Job drawing, mm, ordinate dimensions from the low corner. One solid piece. A direction names the side the tool comes from. Give positions to 0.01 mm unless a question says otherwise; leave off trailing zeros. Order: outer loops, then holes, each group sorted by start corner. A loop starts at its lowest first (then second) coordinate and runs counter-clockwise, first axis right, second up. Notation, with made-up numbers: (-13, 29) - (37, 29) arc R20 cw to (37, 49) - close; hole circle Ø8 at (-37, 6). An arc over 180 degrees is marked (long way). One line per item, written item: value.
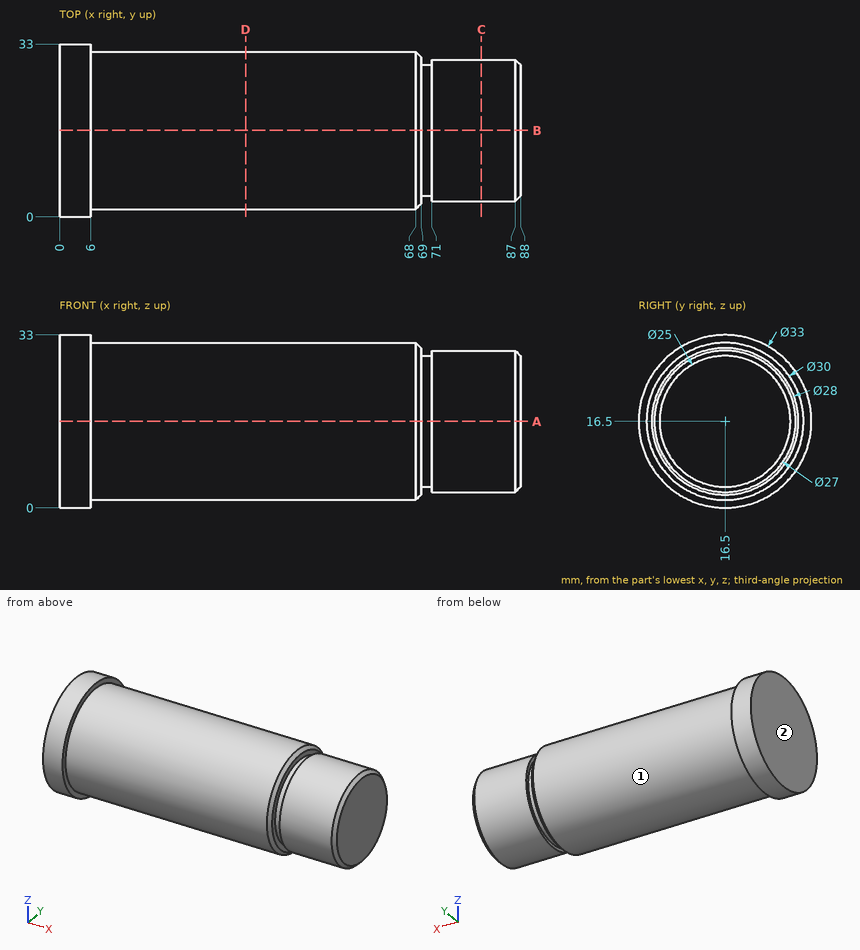
1) Slice it at C-C on x = 80.5. Write the cut outline in (y, z).
Answer:
outline: circle Ø27 at (16.5, 16.5)
2) Slice it at A-A on z = 16.5. Write the cut outline in (x, y).
Answer:
outline: (0, 0) - (6, 0) - (6, 1.5) - (68, 1.5) - (69, 2.5) - (69, 4) - (71, 4) - (71, 3) - (87, 3) - (88, 4) - (88, 29) - (87, 30) - (71, 30) - (71, 29) - (69, 29) - (69, 30.5) - (68, 31.5) - (6, 31.5) - (6, 33) - (0, 33) - close
3) Which spindle directions (+Z, -Z, +X, -X, +Y, -Y) get a long thin tool onto all of the face, cutting with end or side? Do the marked faces 1 and 2. Say none if no direction does.
Answer:
face 1: +X
face 2: +Z, -Z, -X, +Y, -Y
4) Wall check: line 1 along Y through (x, z) = (78.5, 16); line 2 along Y through (x, z) = (15.5, 17); line 3 along Z through (x, y) = (50, 17.5). Give the ranges that are in metal, low to high. Write a range as [from, to].
Answer:
line 1: y = [3.01, 29.99]
line 2: y = [1.51, 31.49]
line 3: z = [1.53, 31.47]
5) Slice it at D-D on x = 35.5. Write the cut outline in (y, z).
Answer:
outline: circle Ø30 at (16.5, 16.5)
6) Drop flat-ended pins along their axis: P1, Ø8, axis at x = 45.5, y = 20.5, coming from the +Z side; P2, Ø2, axis at x = 20, y = 18.5, coming from the -Z side; P3, Ø2, axis at x = 16, z = 24.5, coming from the +Y side. Give the stop position or say it passes through.
Answer:
P1: stops at z = 31.5
P2: stops at z = 1.53
P3: stops at y = 29.77
